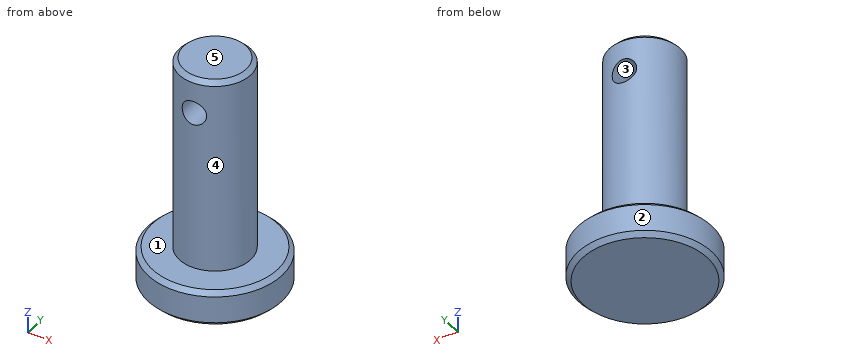
```python
from build123d import *

# Parameters (mm, degrees)
SKETCH1_R               = 4
BOSS_EXTRUDE1_DEPTH     = 22
SKETCH2_R               = 7.5
BOSS_EXTRUDE2_DEPTH     = 4
CUT_EXTRUDE1_DEPTH      = 25.423349484
CUT_EXTRUDE1_DEPTH_BACK = 25.423349484
SKETCH3_R               = 1.35
CHAMFER1_SIZE           = 0.5


with BuildPart() as part:
    # Sketch1 → Boss-Extrude1 (new body)
    with BuildSketch(Plane.XY):
        Circle(SKETCH1_R)
    extrude(amount=BOSS_EXTRUDE1_DEPTH)

    # Sketch2 → Boss-Extrude2 (add)
    with BuildSketch(Plane(origin=(0, 0, 0), x_dir=(-1, 0, 0), z_dir=(0, 0, -1))):
        Circle(SKETCH2_R)
    extrude(amount=BOSS_EXTRUDE2_DEPTH)

    # Sketch3 → Cut-Extrude1 (cut, two sides: drawn at the far end of the back side and taken through both)
    with BuildSketch(Plane(origin=(0, 0, 0), x_dir=(1, 0, 0), z_dir=(0, 1, 0)).offset(-CUT_EXTRUDE1_DEPTH_BACK)):
        with Locations(Location((0, -18, 0), (0, 0, 270))):
            Circle(SKETCH3_R)
    extrude(amount=CUT_EXTRUDE1_DEPTH + CUT_EXTRUDE1_DEPTH_BACK, mode=Mode.SUBTRACT)

    # Chamfer1
    chamfer1_edges = [part.edges().sort_by_distance(p)[0] for p in [
        (-4, 0, 22),
        (7.5, 0, 0),
        (7.5, 0, -4),
    ]]
    chamfer(chamfer1_edges, length=CHAMFER1_SIZE)


solid = part.part
```
The model under review builds one solid part; all positions refer to its coordinate system, in mm. Face numbers are marked on the shaded views. A direction names the side the tool comes from. Round coordinates to 2 decimals unless told otherwise and drop trailing zeros. Order: outer loops, then holes, each group sorted by start corner. A loop starts at its lowest first (then second) coordinate and runs counter-clockwise, first axis right, second up. Notation, with made-up numbers: (45.5, 89.5) -> (50.5, 89.5) arc R23 ccw to (50.5, 109.5) -> close; hole circle Ø8 at (18, 78). An arc over 180 degrees is marked (long way). One line per item, written item: value. Start each with the question number.
Q1. Machinability: for the marked faces 4 and 5, which of the approach directions +Z, -Z, +X, -X, +Y, -Y give a long, thin tool a straight path to every point of the face, cutting with its end or side? Answer none if there is none.
Q2. Take a section at D-D (z = 14). Write out the cut boundary in (x, y), and give its area (3 significant figures).
Q3. Take a section at A-A (y = 0). Write out the cut boundary in (x, z).
Q4. Take a section at B-B (x = 0). Write out the cut boundary in (y, z).
Q5. Clearance check with flat-ended pins moving along their axes: pin 1 Ø2 at (x, z) = (1, 1.5) entering from -Y; pin 2 Ø2 at (y, z) = (-0.5, 14.5) entering from -X; pin 3 Ø1 at (y, z) = (4, 2) entering from +X. State where each tip first meets the part, or that it passes through.
Q6. Wall thickness on line 1 (Z direction, x = 0, y = -0.25); line 2 (Z direction, x = -4.5, y = 1); line 3 (X direction, y = -1, z = 18): over which ranges is each line inside the solid? List them lowest first.
Q7. Take a section at C-C (z = 18.75). Write out the cut boundary in (x, y).
Q8. Mouldability with a two-part tool opening along Z and no side actions: class the marked faces 1, 2 and 3 as released by +Z, released by -Z, zero draft, split by the parting line, or undercut.
Reported:
1. face 4: +Z
1. face 5: +Z, +X, -X, +Y, -Y
2. outline: circle Ø8 at (0, 0)
2. area: 50.3 mm2
3. outline: (-7.5, -3.5) -> (-7, -4) -> (7, -4) -> (7.5, -3.5) -> (7.5, -0.5) -> (7, 0) -> (4, 0) -> (4, 21.5) -> (3.5, 22) -> (-3.5, 22) -> (-4, 21.5) -> (-4, 0) -> (-7, 0) -> (-7.5, -0.5) -> close; hole circle Ø2.7 at (0, 18)
4. outline: (-7.5, -3.5) -> (-7, -4) -> (7, -4) -> (7.5, -3.5) -> (7.5, -0.5) -> (7, 0) -> (4, 0) -> (4, 16.65) -> (-4, 16.65) -> (-4, 0) -> (-7, 0) -> (-7.5, -0.5) -> close; (-4, 19.35) -> (4, 19.35) -> (4, 21.5) -> (3.5, 22) -> (-3.5, 22) -> (-4, 21.5) -> close
5. pin 1: stops at y = -4
5. pin 2: stops at x = -4
5. pin 3: stops at x = 1.94
6. line 1: z = -4 to 16.65, 19.35 to 22
6. line 2: z = -4 to 0
6. line 3: x = -3.87 to -1.35, 1.35 to 3.87
7. outline: (-1.12, -3.84) -> (-1.12, 3.84) arc R4 ccw to start; (1.12, -3.84) arc R4 ccw to (1.12, 3.84) -> close
8. face 1: released by +Z
8. face 2: zero draft
8. face 3: undercut
